Geometry: final body of the model. Coordinates: model frame, mm. A direction names the side the tool comes from. Coordinates: 2 decimals unless noted, no trailing zeros. Loops run counter-clockwise (first coordinate to the right, second up) from the corner with the lowest first, then second, coordinate; pieces in that order, holes last. Notation, with made-up numbers: (-29.5, 17.25) - (-8.5, 17.25) arc R13 ccw to (-8.5, 25.25) - close; hole circle Ø11 at (48, 8.5). An arc over 180 degrees is marked (long way). Answer in a Markdown table with one row per item.
from build123d import *

# Parameters (mm, degrees)
BASE_BLOCK_DEPTH      = 75
BOTTOM_NOTCH_SKETCH_W = 35
BOTTOM_NOTCH_SKETCH_H = 40
BOTTOM_NOTCH_DEPTH    = 155.029218007
TOP_SLOT_SKETCH_W     = 45
TOP_SLOT_SKETCH_H     = 90
TOP_SLOT_DEPTH        = 40
EDGE_FILLET_R18_R     = 18
CROSS_HOLE_SKETCH_R   = 10
CROSS_HOLE_DEPTH      = 155.029218007
PIN_HOLE_SKETCH_R     = 12.5
PIN_HOLE_DEPTH        = 40
SIDE_LUGS_SKETCH_R    = 8
SIDE_LUGS_DEPTH       = 15


with BuildPart() as part:
    # Base Profile Sketch → Base Block (new body)
    with BuildSketch(Plane(origin=(0, 0, 0), x_dir=(0, 0, -1), z_dir=(1, 0, 0))):
        Polygon((0, 0), (90, 0), (90, 60), (45, 100), (0, 100), align=None)
    extrude(amount=-BASE_BLOCK_DEPTH)

    # Bottom Notch Sketch → Bottom Notch (cut, through all)
    with BuildSketch(Plane(origin=(0, 0, -90), x_dir=(-1, 0, 0), z_dir=(0, 0, -1))):
        with Locations((37.5, 20)):
            Rectangle(BOTTOM_NOTCH_SKETCH_W, BOTTOM_NOTCH_SKETCH_H)
    extrude(amount=-BOTTOM_NOTCH_DEPTH, mode=Mode.SUBTRACT)

    # Top Slot Sketch → Top Slot (cut)
    with BuildSketch(Plane(origin=(0, 100, 0), x_dir=(1, 0, 0), z_dir=(0, 1, 0))):
        with Locations((-37.5, 45)):
            Rectangle(TOP_SLOT_SKETCH_W, TOP_SLOT_SKETCH_H)
    extrude(amount=-TOP_SLOT_DEPTH, mode=Mode.SUBTRACT)

    # Edge Fillet R18
    edge_fillet_r18_edges = [part.edges().sort_by_distance(p)[0] for p in [
        (-7.5, 100, -45),
        (-67.5, 100, -45),
    ]]
    fillet(edge_fillet_r18_edges, radius=EDGE_FILLET_R18_R)

    # Cross Hole Sketch → Cross Hole (cut, through all)
    with BuildSketch(Plane(origin=(0, 0, 0), x_dir=(0, 0, -1), z_dir=(1, 0, 0))):
        with Locations((35, 80)):
            Circle(CROSS_HOLE_SKETCH_R)
    extrude(amount=-CROSS_HOLE_DEPTH, mode=Mode.SUBTRACT)

    # Pin Hole Sketch → Pin Hole (cut)
    with BuildSketch(Plane(origin=(0, 60, 0), x_dir=(1, 0, 0), z_dir=(0, 1, 0))):
        with Locations(Location((-37.5, 76, 0), (0, 0, 270))):
            Circle(PIN_HOLE_SKETCH_R)
    extrude(amount=-PIN_HOLE_DEPTH, mode=Mode.SUBTRACT)

    # Side Lugs Sketch → Side Lugs (add)
    # profile 1 of 2: a face of its own
    with BuildSketch(Plane.XY):
        with BuildLine():
            Line((15, 72), (0, 72))
            Line((0, 72), (0, 0))
            Line((0, 0), (25.855763811, 54.886059047))
            ThreePointArc((25.855763811, 54.886059047), (25.133293922, 66.427779888), (15, 72))
        make_face()
        with Locations((15, 60)):
            Circle(SIDE_LUGS_SKETCH_R, mode=Mode.SUBTRACT)
    # profile 2 of 2: a face of its own
    with BuildSketch(Plane.XY):
        with BuildLine():
            Line((-90, 72), (-75, 72))
            Line((-75, 72), (-75, 0))
            Line((-75, 0), (-100.855763811, 54.886059047))
            ThreePointArc((-100.855763811, 54.886059047), (-100.133293922, 66.427779888), (-90, 72))
        make_face()
        with Locations((-90, 60)):
            Circle(SIDE_LUGS_SKETCH_R, mode=Mode.SUBTRACT)
    extrude(amount=-SIDE_LUGS_DEPTH)


solid = part.part
(1) Cut plane A-A on z = -7. Output: boundary loops of the cut face in (x, y), then the cut area to 3 significant figures.
Verdict:
| item | result |
|---|---|
| outline | (-100.86, 54.89) - (-75, 0) - (-55, 0) - (-55, 40) - (-20, 40) - (-20, 0) - (0, 0) - (25.86, 54.89) arc R12 ccw to (15, 72) - (0, 72) - (0, 100) - (-15, 100) - (-15, 60) - (-60, 60) - (-60, 100) - (-75, 100) - (-75, 72) - (-90, 72) arc R12 ccw to start; hole circle Ø16 at (-90, 60); hole circle Ø16 at (15, 60) |
| area | 6,180 mm² |
(2) Access query for faces 1 (the face through (-20, 20, -46)), 2 (the face through (-100.223, 66.284, -7.395)), 3 (the face through (-38, 60, -46)). Directions: +Z, -Z, +X, -X, +Y, -Y. A direction counts if a zero-diameter tool reaches every point of the face in a straight line with its end or side. Return the directions, or none.
Verdict:
| item | result |
|---|---|
| face 1 | +Z, -Z, -Y |
| face 2 | +Z, -Z, -X |
| face 3 | +Z, -Z, +Y |
(3) Cut plane D-D on z = -19.5. Output: boundary loops of the cut face in (x, y).
Verdict:
| item | result |
|---|---|
| outline | (-75, 0) - (-55, 0) - (-55, 40) - (-20, 40) - (-20, 0) - (0, 0) - (0, 100) - (-15, 100) - (-15, 60) - (-60, 60) - (-60, 100) - (-75, 100) - close |
(4) Cut plane C-C on y = 80. Output: boundary loops of the cut face in (x, z).
Verdict:
| item | result |
|---|---|
| outline | (-75, -67.5) - (-60, -67.5) - (-60, -45) - (-75, -45) - close; (-75, -25) - (-60, -25) - (-60, 0) - (-75, 0) - close; (-15, -67.5) - (0, -67.5) - (0, -45) - (-15, -45) - close; (-15, -25) - (0, -25) - (0, 0) - (-15, 0) - close |
(5) First-contact query: pin 1 Ø20 at (y, z) = (11.5, -51) entering from +X; pin 2 Ø20 at (y, z) = (88, -61.5) entering from -X; pin 3 Ø21.5 at (x, y) = (-90, 38.5) entering from -Z; pin 4 Ø5 at (y, z) = (80.5, -71) entering from -X. Flat tips, straight axial feed; report the tip coordinate or a pass-through.
Verdict:
| item | result |
|---|---|
| pin 1 | stops at x = 0 |
| pin 2 | stops at x = -75 |
| pin 3 | stops at z = -15 |
| pin 4 | passes through |
(6) Cut plane B-B on x = -37.5. Output: boundary loops of the cut face in (y, z).
Verdict:
| item | result |
|---|---|
| outline | (40, -90) - (60, -90) - (60, -88.5) - (40, -88.5) - close; (40, -63.5) - (60, -63.5) - (60, 0) - (40, 0) - close |
(7) Pull-direction query (Y, two-part tool) for faces 4 (the face through (-65, 0, -44)), 5 (the face through (-7.395, 89.915, -33.698)), 6 (the face through (-85, 45, -15)); classes: pulls with the +Y half, pulls with the -Y half, needs draft (parallel to the pull), parting line crosses it, or undercut.
Verdict:
| item | result |
|---|---|
| face 4 | pulls with the -Y half |
| face 5 | undercut |
| face 6 | needs draft |
(8) Ray query, probe 1 along X at (y, z) = (12, -71.5); probe 2 along X at (y, z) = (63.5, -19); probe 3 along Y at (x, z) = (-64.5, -35). Return the intervals inside material, ascending.
Verdict:
| item | result |
|---|---|
| probe 1 | x = -75 to -55, -20 to 0 |
| probe 2 | x = -75 to -60, -15 to 0 |
| probe 3 | y = 0 to 70, 90 to 100 |
